Here's how the part is built. I have some questions about the finished solid (model axes, mm). Face numbers are marked on the shaded views. Round coordinates to 2 decimals unless told otherwise and drop trailing zeros. Order: outer loops, then holes, each group sorted by start corner. A loop starts at its lowest first (then second) coordinate and runs counter-clockwise, first axis right, second up. Notation, with made-up numbers: (-1.75, 22) -> (40.25, 22) arc R28 cw to (40.25, 59) -> close; hole circle Ø10 at (76.5, -38). An arc over 180 degrees is marked (long way). Answer in a Markdown table with one row per item.
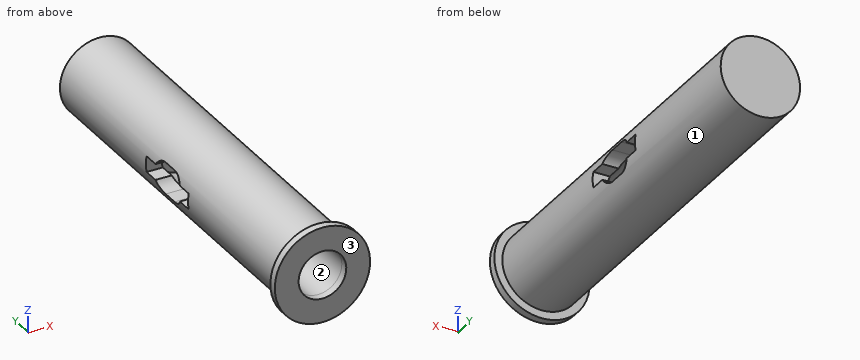
```python
from build123d import *

# Parameters (mm, degrees)
CUT_EXTRUDE1_DEPTH  = 52.23475383
SKETCH9_R           = 6
SKETCH9_R_2         = 3
BOSS_EXTRUDE3_DEPTH = 1
CUT_EXTRUDE2_DEPTH  = 52.546095972


with BuildPart() as part:
    # Sketch3 → Revolve1 (revolve)
    with BuildSketch(Plane.XY, mode=Mode.PRIVATE) as revolve1_sk:
        Polygon((3.025, 0), (3.025, 32.1), (0, 32.1), (0, 50), (5, 50), (5, 0), align=None)
    revolve(revolve1_sk.sketch.rotate(Axis((0, -0.72972973, 0), (0, 1, 0)), 90), axis=Axis((0, -0.72972973, 0), (0, 1, 0)))

    # Sketch6 → Cut-Extrude1 (cut, through all)
    with BuildSketch(Plane(origin=(5, 0, 0), x_dir=(0, 0, -1), z_dir=(1, 0, 0))):
        with BuildLine():
            Line((2, 27), (2, 25))
            ThreePointArc((2, 25), (0, 23), (-2, 25))
            Line((-2, 25), (-2, 27))
            ThreePointArc((-2, 27), (0, 29), (2, 27))
        make_face()
    extrude(amount=-CUT_EXTRUDE1_DEPTH, mode=Mode.SUBTRACT)

    # Sketch9 → Boss-Extrude3 (add)
    with BuildSketch(Plane(origin=(0, 0, 0), x_dir=(1, 0, 0), z_dir=(0, 1, 0))):
        with Locations(Location((0, 0, 0), (0, 0, 270))):
            Circle(SKETCH9_R)
        with Locations(Location((0, 0, 0), (0, 0, 270))):
            Circle(SKETCH9_R_2, mode=Mode.SUBTRACT)
    extrude(amount=BOSS_EXTRUDE3_DEPTH)

    # Sketch11 → Cut-Extrude2 (cut, through all)
    with BuildSketch(Plane(origin=(5, 0, 0), x_dir=(0, 0, -1), z_dir=(1, 0, 0))):
        Polygon((-1, 23.267949192), (-1, 21.267949192), (1, 21.267949192), (1, 23.267949192), (1, 28.732050808), (1, 30.732050808), (-1, 30.732050808), (-1, 28.732050808), align=None)
    extrude(amount=-CUT_EXTRUDE2_DEPTH, mode=Mode.SUBTRACT)


solid = part.part
```
1. Suppose I cut it at A-A on z = 0. Write out the boundary of the cut face in (x, y) (3 decimals).
Numbers:
| item | result |
|---|---|
| outline | (-6, 0) -> (-3, 0) -> (-3, 1) -> (-3.025, 1) -> (-3.025, 21.268) -> (-5, 21.268) -> (-5, 1) -> (-6, 1) -> close; (-5, 30.732) -> (-3.025, 30.732) -> (-3.025, 32.1) -> (3.025, 32.1) -> (3.025, 30.732) -> (5, 30.732) -> (5, 50) -> (-5, 50) -> close; (3, 0) -> (6, 0) -> (6, 1) -> (5, 1) -> (5, 21.268) -> (3.025, 21.268) -> (3.025, 1) -> (3, 1) -> close |
2. Suppose I cut it at C-C on z = 3.5. Write out the boundary of the cut face in (x, y), then the cut area to 3 significant figures.
Numbers:
| item | result |
|---|---|
| outline | (-4.87, 0) -> (4.87, 0) -> (4.87, 1) -> (3.57, 1) -> (3.57, 50) -> (-3.57, 50) -> (-3.57, 1) -> (-4.87, 1) -> close |
| area | 360 mm2 |
3. Please list where these lines run through material, in increasing order: line 1 along X through (y, z) = (12, 0) (3 decimals); line 2 along X through (y, z) = (0.4, 0); line 3 along Y through (x, z) = (-1, 1.5).
Numbers:
| item | result |
|---|---|
| line 1 | x = -5 to -3.025, 3.025 to 5 |
| line 2 | x = -6 to -3, 3 to 6 |
| line 3 | y = 32.1 to 50 |
4. Suppose I cut it at D-D on y = 43. Write out the boundary of the cut face in (x, z), then the cut area to 3 significant figures.
Numbers:
| item | result |
|---|---|
| outline | circle Ø10 at (0, 0) |
| area | 78.5 mm2 |
5. For pin 1 Ø4 at (y, z) = (23, 0.5) entering from -X; pin 2 Ø2 at (x, y) = (4.5, 30) entering from +Z; pin 3 Ø1.8 at (x, z) = (1.5, 0.5) entering from -Y; pin 4 Ø1.6 at (x, z) = (4, -0.5) entering from -Y, each with a flat end and sliding along its axis, tell me the tip position at first contact or that it passes through.
Numbers:
| item | result |
|---|---|
| pin 1 | stops at x = -5 |
| pin 2 | stops at z = 3.57 |
| pin 3 | stops at y = 32.1 |
| pin 4 | stops at y = 0 |
6. We'd pull the mould along X, two halves only. Please class the marked faces 1, 2 and 3: released by +X, released by -X, zero draft, split by the parting line, or undercut.
Numbers:
| item | result |
|---|---|
| face 1 | split by the parting line |
| face 2 | undercut |
| face 3 | zero draft |
